```python
from build123d import *

# Parameters (mm, degrees)
CHAMFER1_SIZE  = 2
CHAMFER1_SIZE2 = 6


with BuildPart() as part:
    # Sketch1 → Revolve1 (revolve)
    with BuildSketch(Plane.XY, mode=Mode.PRIVATE) as revolve1_sk:
        Polygon((0, 7.5), (0, 15), (105, 15), (105, 12), (183, 12), (183, 7.5), (33, 7.5), (33, 3.25), (8, 3.25), (8, 7.5), align=None)
    revolve(revolve1_sk.sketch.rotate(Axis((0, 0, 0), (1, 0, 0)), 90), axis=Axis((0, 0, 0), (1, 0, 0)))

    # Chamfer1
    chamfer1_edges = [part.edges().sort_by_distance(p)[0] for p in [
        (183, 0, -12),
    ]]
    chamfer1_side = [part.faces().sort_by_distance(p)[0] for p in [
        (183, 0, -11.660588745),
    ]]
    chamfer(chamfer1_edges, length=CHAMFER1_SIZE, length2=CHAMFER1_SIZE2, reference=chamfer1_side[0])


solid = part.part
```
Design review of the part built by this model. Coordinates are the model's own, in mm. A direction names the side the tool comes from. Round coordinates to 2 decimals unless told otherwise and drop trailing zeros. Order: outer loops, then holes, each group sorted by start corner. A loop starts at its lowest first (then second) coordinate and runs counter-clockwise, first axis right, second up. Notation, with made-up numbers: (76, 41.5) - (100, 41.5) arc R31 cw to (100, 68.5) - close; hole circle Ø4 at (58, 66). An arc over 180 degrees is marked (long way). Return JSON: item names as keys, results as strings.
Q1. Wall thickness on L1, parallel to Y at x = 27.5, z = 0; L2, parallel to Y at x = 90, z = 0; L3, parallel to X at y = 1.5, z = -6.5: over which ranges is each line inside the solid? List them lowest first. Write a range as [from, to].
Computed values:
{"L1": "y = [-15, -3.25], [3.25, 15]", "L2": "y = [-15, -7.5], [7.5, 15]", "L3": "x = [8, 33]"}
Q2. Machinability: for faces 1 (the flat face through (33, 3, 2)), 2 (the cylindrical face through (53.24, -12.65, 8.06)), which of the approach directions +Z, -Z, +X, -X, +Y, -Y give a long, thin tool a straight path to every point of the face, cutting with its end or side? Answer none if there is none.
Computed values:
{"face 1": "+X", "face 2": "+X, -X"}
Q3. For pin 1 Ø6 at (y, z) = (0, 0) entering from -X; pin 2 Ø8 at (x, z) = (88, 9.5) entering from +Y; pin 3 Ø1.5 at (x, y) = (135.5, -1) entering from +Z; pin 4 Ø1 at (y, z) = (-4, -2) entering from -X, all flat-tipped, find the tip position at first contact; note any pin that passes through.
Computed values:
{"pin 1": "passes through", "pin 2": "stops at y = 13.96", "pin 3": "stops at z = 12", "pin 4": "stops at x = 8"}
Q4. Consider section A-A on y = 0. Write out the cut boundary in (x, z), plus the area to 3 significant figures.
Computed values:
{"outline": "(0, -15) - (105, -15) - (105, -12) - (177, -12) - (183, -10) - (183, -7.5) - (33, -7.5) - (33, -3.25) - (8, -3.25) - (8, -7.5) - (0, -7.5) - close; (0, 7.5) - (8, 7.5) - (8, 3.25) - (33, 3.25) - (33, 7.5) - (183, 7.5) - (183, 10) - (177, 12) - (105, 12) - (105, 15) - (0, 15) - close", "area": "2,480 mm2"}
Q5. Consider section C-C on x = 158.5. Write out the cut boundary in (y, z), plus the area to 3 significant figures.
Computed values:
{"outline": "circle Ø24 at (0, 0); hole circle Ø15 at (0, 0)", "area": "276 mm2"}
Q6. The part is to be moulded in two halves that separate along Z. For faces 3 (the flat face through (183, -7, 4)), 4 (the cylindrical face through (141.504, -3.604, 11.446)), 5 (the flat face through (8, 2, -3)), 6 (the cylindrical face through (3.944, -6.324, 4.032)), say which applies: pulls with the +Z half, pulls with the -Z half, needs draft (parallel to the pull), parting line crosses it, or undercut.
Computed values:
{"face 3": "needs draft", "face 4": "parting line crosses it", "face 5": "undercut", "face 6": "undercut"}
Q7. Consider section D-D on x = 84. Write out the cut boundary in (y, z).
Computed values:
{"outline": "circle Ø30 at (0, 0); hole circle Ø15 at (0, 0)"}
